from build123d import *

# Parameters (mm, degrees)
SKETCH1_R           = 4
BOSS_EXTRUDE1_DEPTH = 10


with BuildPart() as part:
    # Sketch1 → Boss-Extrude1 (new body)
    with BuildSketch(Plane.XY):
        with BuildLine():
            Line((0, 7.5), (69, 7.5))
            ThreePointArc((69, 7.5), (74.303300859, 5.303300859), (76.5, 0))
            Line((76.5, 0), (60.5, 0))
            Line((60.5, 0), (55.535633926, -7.5))
            Line((55.535633926, -7.5), (0, -7.5))
            ThreePointArc((0, -7.5), (-7.5, 0), (0, 7.5))
        make_face()
        Circle(SKETCH1_R, mode=Mode.SUBTRACT)
    extrude(amount=BOSS_EXTRUDE1_DEPTH)


solid = part.part
Check sheet for the modelled part. Datum: model origin and axes. Units: mm. Give positions to 0.01 mm unless a question says otherwise; leave off trailing zeros. Write each loop counter-clockwise with the first axis right and the second up, starting at its lowest first coordinate (ties: lowest second). Pieces come first, ordered by that corner, then holes. Notation, with made-up numbers: (30, 49.5) -> (88, 49.5) arc R17 ccw to (88, 54.5) -> close; hole circle Ø9 at (-17, -5.5). An arc over 180 degrees is marked (long way). One line per item, written item: value. Start each with the question number.
Item 1: Section check A-A on z = 1. Record the cut outline in (x, y), then the cut area to 3 significant figures.
Item 2: Material ranges on probe 1 along Y at (x, z) = (0, 2.5); probe 2 along X at (y, z) = (-0.5, 7.75); probe 3 along X at (y, z) = (-3.5, 5.75), recorded low to high. Write a range as from..to.
Item 3: Draft check along Y on faces 1 (the flat face through (69, 0, 5)), 2 (the cylindrical face through (-0.867, -3.905, 4.93)), 3 (the flat face through (35, 0, 10)). Enter one of: +Y half, -Y half, draft (parallel to the pull), parting line (faces both ways), or undercut.
Item 4: Section check B-B on y = 3. Record the cut outline in (x, z), then the cut area to 3 significant figures.
Item 5: Section check C-C on y = -1. Record the cut outline in (x, z).
Item 6: Section check D-D on y = -5.5. Record the cut outline in (x, z), then the cut area to 3 significant figures.
Item 7: Gauge pin test, flat ends, axial feed: pin 1 (2 mm diameter, centred on x = 57, z = 4, fed in from -Y); pin 2 (6.5 mm diameter, centred on x = 0, y = 0, fed in from -Z); pin 3 (5 mm diameter, centred on x = 71, z = 2.5, fed in from -Y); pin 4 (6 mm diameter, centred on y = -3.5, z = 2.5, fed in from +X). Record the tip position at first contact, or that the pin passes through.
Results list:
1. outline: (0, -7.5) -> (55.54, -7.5) -> (60.5, 0) -> (76.5, 0) arc R7.5 ccw to (69, 7.5) -> (0, 7.5) arc R7.5 ccw to start; hole circle Ø8 at (0, 0)
1. area: 1,030 mm²
2. probe 1: -7.5..-4, 4..7.5
2. probe 2: -7.48..-3.97, 3.97..60.17
2. probe 3: -6.63..-1.94, 1.94..58.18
3. face 1: -Y half
3. face 2: undercut
3. face 3: draft
4. outline: (-6.87, 0) -> (-2.65, 0) -> (-2.65, 10) -> (-6.87, 10) -> close; (2.65, 0) -> (75.87, 0) -> (75.87, 10) -> (2.65, 10) -> close
4. area: 775 mm²
5. outline: (-7.43, 0) -> (-3.87, 0) -> (-3.87, 10) -> (-7.43, 10) -> close; (3.87, 0) -> (59.84, 0) -> (59.84, 10) -> (3.87, 10) -> close
6. outline: (-5.1, 0) -> (56.86, 0) -> (56.86, 10) -> (-5.1, 10) -> close
6. area: 620 mm²
7. pin 1: y = -6.8
7. pin 2: through
7. pin 3: y = 0
7. pin 4: x = 60.17
